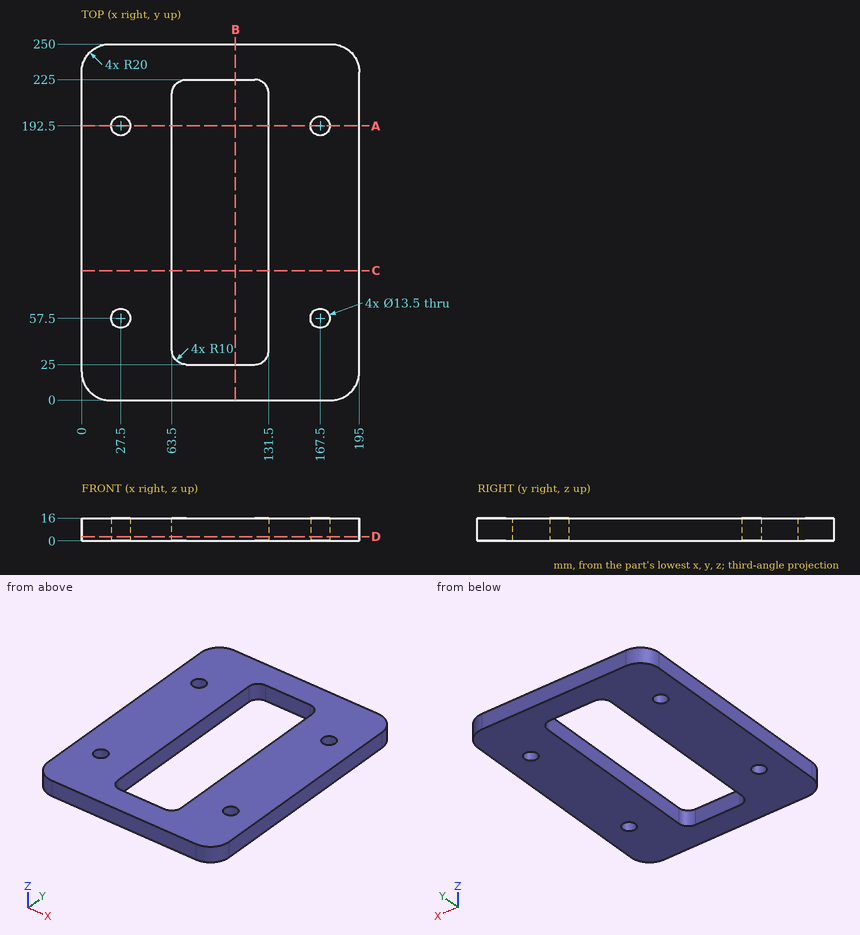
Part print with two shaded views. Sizes in mm from the minimum x, y, z corner. Give positions to 0.01 mm unless a question says otherwise; leave off trailing zeros. Order: outer loops, then holes, each group sorted by start corner. A loop starts at its lowest first (then second) coordinate and runs counter-clockwise, first axis right, second up. Notation, with made-up numbers: M -12,52 L 43,52 A32 ccw 43,78 Z; hole C 61.25,-15.5 d3. An arc over 180 degrees is marked long. Write item = value, one per line.
Q1. Cut at B-B, the plane x = 108. List the corners of the cut face in (y, z), then the cut area to 3 significant figures.
Derived:
outline = M 0,0 L 25,0 L 25,16 L 0,16 Z; M 225,0 L 250,0 L 250,16 L 225,16 Z
area = 800 mm2
Q2. Drill centre lines: line 1 (Y direction, x = 167.5, z = 12.5); line 2 (X direction, y = 145.5, z = 11.25); line 3 (Y direction, x = 103.5, z = 5.75). Where is each one in solid material? Low to high. Write a range as [from, to].
Derived:
line_1 = [0, 50.75], [64.25, 185.75], [199.25, 250]
line_2 = [0, 63.5], [131.5, 195]
line_3 = [0, 25], [225, 250]
Q3. Cut at A-A, the plane y = 192.5. List the corners of the cut face in (x, z).
Derived:
outline = M 0,0 L 20.75,0 L 20.75,16 L 0,16 Z; M 34.25,0 L 63.5,0 L 63.5,16 L 34.25,16 Z; M 131.5,0 L 160.75,0 L 160.75,16 L 131.5,16 Z; M 174.25,0 L 195,0 L 195,16 L 174.25,16 Z
Q4. Cut at C-C, the plane y = 91. List the corners of the cut face in (x, z), then the cut area to 3 significant figures.
Derived:
outline = M 0,0 L 63.5,0 L 63.5,16 L 0,16 Z; M 131.5,0 L 195,0 L 195,16 L 131.5,16 Z
area = 2,030 mm2
Q5. Cut at D-D, the plane z = 3. List the corners of the cut face in (x, y), then the cut area to 3 significant figures.
Derived:
outline = M 0,20 A20 ccw 20,0 L 175,0 A20 ccw 195,20 L 195,230 A20 ccw 175,250 L 20,250 A20 ccw 0,230 Z; hole C 27.5,57.5 d13.5; hole C 27.5,192.5 d13.5; hole M 63.5,35 A10 ccw 73.5,25 L 121.5,25 A10 ccw 131.5,35 L 131.5,215 A10 ccw 121.5,225 L 73.5,225 A10 ccw 63.5,215 Z; hole C 167.5,57.5 d13.5; hole C 167.5,192.5 d13.5
area = 34,300 mm2
Q6. Flat gauge pin, fed straight in: pin 1 (4 mm diameter, centred on y = 35, z = 9, fed in from -X). Where does the tip first touch, or does it go through?
Derived:
pin_1 = 0
